Check sheet for the modelled part. Datum: model origin and axes. Units: mm. A direction names the side the tool comes from. Round coordinates to 2 decimals unless told otherwise and drop trailing zeros. Loops run counter-clockwise (first coordinate to the right, second up) from the corner with the lowest first, then second, coordinate; pieces in that order, holes last. Notation, with made-up numbers: (35.25, 49) -> (45.25, 49) arc R23 cw to (45.25, 85) -> close; hole circle Ø11 at (7, -21). An arc over 180 degrees is marked (long way). One line per item, written item: value. Start each with the question number.
1. Cross-section at D-D on x = 22. Record the cut outline in (y, z), then the cut area to 3 significant figures.
2. Material ranges on L1, parallel to X at y = -124, z = -19; L2, parallel to X at y = -44.5, z = 3; L3, parallel to Z at x = 19, y = 68, recorded low to high.
3. Cross-section at B-B on z = -18. Record the cut outline in (x, y).
4. Go/stop test with flat-tipped pins: pin 1 (2 mm diameter, centred on x = 4, y = 110, fed in from -Z); pin 2 (9 mm diameter, centred on y = -83, z = -13.5, fed in from -X); pin 3 (15 mm diameter, centred on y = -147, z = -17, fed in from +X). Record where each tip stops, or that it passes through.
5. Set-up check for faces 4 (the face through (-55, 33.599, -12)), 5 (the face through (-55, -121, -25)): record each of +Z, -Z, +X, -X, +Y, -Y from which the full face is reachable in a straight line by a thin tool's end or side.
6. Cross-section at A-A on y = -163. Record the cut outline in (x, z), then the cut area to 3 significant figures.
7. Cross-section at C-C on y = -30. Record the cut outline in (x, z), then the cut area to 3 significant figures.
8. Release check for a two-part mould opening along X. For faces 1 (the face through (-50, -125, -10)), 2 (the face through (55, 5.758, -12)), 3 (the face through (60, -122, -10)) record: +X half, -X half, draft (parallel to the pull), parting line (faces both ways), or undercut.
from build123d import *

# Parameters (mm, degrees)
BOSS_EXTRUDE1_DEPTH = 5
SKETCH2_W           = 10
SKETCH2_H           = 285.757818937
SKETCH2_H_2         = 313.599020197
BOSS_EXTRUDE2_DEPTH = 30
CHAMFER1_SIZE       = 3.5


with BuildPart() as part:
    # Sketch1 → Boss-Extrude1 (new body)
    with BuildSketch(Plane.XY):
        Polygon((-60, 40), (-60, -80), (60, -80), (60, 40), (70, 40), (70, 190), (-80, 190), (-80, 40), align=None)
    extrude(amount=BOSS_EXTRUDE1_DEPTH)

    # Sketch2 → Boss-Extrude2 (add)
    with BuildSketch(Plane.XY.offset(5)):
        with Locations((55, -137.121090531)):
            Rectangle(SKETCH2_W, SKETCH2_H)
        with Locations((-55, -123.200489901)):
            Rectangle(SKETCH2_W, SKETCH2_H_2)
    extrude(amount=-BOSS_EXTRUDE2_DEPTH)

    # Chamfer1
    chamfer1_edges = [part.edges().sort_by_distance(p)[0] for p in [
        (0, -80, 5),
    ]]
    chamfer(chamfer1_edges, length=CHAMFER1_SIZE)


solid = part.part
Taken from the geometry:
1. outline: (-80, 0) -> (190, 0) -> (190, 5) -> (-76.5, 5) -> (-80, 1.5) -> close
1. area: 1,340 mm2
2. L1: x = -60 to -50, 50 to 60
2. L2: x = -60 to 60
2. L3: z = 0 to 5
3. outline: (-60, -280) -> (-50, -280) -> (-50, 33.6) -> (-60, 33.6) -> close; (50, -280) -> (60, -280) -> (60, 5.76) -> (50, 5.76) -> close
4. pin 1: stops at z = 0
4. pin 2: stops at x = -60
4. pin 3: stops at x = 60
5. face 4: -Z, +X, -X, +Y
5. face 5: -Z, +X, -X, +Y, -Y
6. outline: (-60, -25) -> (-50, -25) -> (-50, 5) -> (-60, 5) -> close; (50, -25) -> (60, -25) -> (60, 5) -> (50, 5) -> close
6. area: 600 mm2
7. outline: (-60, -25) -> (-50, -25) -> (-50, 0) -> (50, 0) -> (50, -25) -> (60, -25) -> (60, 5) -> (-60, 5) -> close
7. area: 1,100 mm2
8. face 1: undercut
8. face 2: draft
8. face 3: +X half
